Input: part model. Units: mm. Frame: model coordinates. Face numbers are marked on the shaded views. A direction names the side the tool comes from. Round coordinates to 2 decimals unless told otherwise and drop trailing zeros. Loops run counter-clockwise (first coordinate to the right, second up) from the corner with the lowest first, then second, coordinate; pieces in that order, holes last. Notation, with made-up numbers: (10, -38) -> (53, -38) arc R23 cw to (53, -11) -> close; hole circle Ø11 at (84, -30). An arc over 180 degrees is marked (long way). Answer as a JSON object with one key per item and string values. Group by question number.
Item 1: Section query C-C on y = 12.75. Count the separate pieces of the cut face and the enclosed holes in it, and give its area (3 significant figures).
Item 2: Draft query along Z for the marked faces 1, 2 and 3. Return one class per face: released by +Z, released by -Z, zero draft, split by the parting line, or undercut.
Item 3: Material intervals for line 1 (X direction, y = 6.75, z = -22); line 2 (Z direction, x = 18, y = 13.25); line 3 (Z direction, x = -18.5, y = 13.5), sorted ascending. Write a range as [from, to].
Item 4: Set-up query: the marked faces 4 and 5. Return all of +Z, -Z, +X, -X, +Y, -Y with unobstructed straight access to the full face (end or side cutting, diameter ignored); none if empty.
Item 5: Section query D-D on z = 27.5. Return loops of the section in (x, y), and give its area (3 significant figures).
Item 6: Pin query (flat end, axial travel): pin 1 (3.5 mm diameter, centred on x = -31.71, z = -10.3, fed in from +Y); pin 2 (13 mm diameter, centred on x = 17.6, z = -24.22, fed in from +Y); pin 3 (2 mm diameter, centred on x = -7.5, y = 11, fed in from -Z); pin 4 (4 mm diameter, centred on y = 14, z = -7, fed in from +X). Return the tip coordinate at first contact, or that it passes through.
Item 7: Section query A-A on z = 0. Return loops of the section in (x, y) (1 decimal), and give its area (3 significant figures).
Item 8: Section query B-B on x = 0. Return loops of the section in (y, z) (1 decimal), and give its area (3 significant figures).
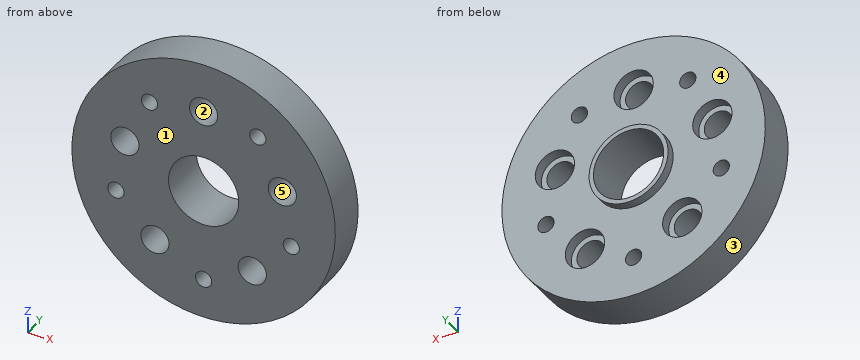
from build123d import *

# Parameters (mm, degrees)
FLANGE_DISC_SKETCH_R              = 47.625
FLANGE_DISC_3_75_DEPTH            = 14.2875
TAPPED_HOLES_SKETCH_R             = 2.930707565
TAPPED_HOLES_5X_ON_BC_2_625_DEPTH = 14.2875
HUB_BOSS_SKETCH_R                 = 14.2875
HUB_BOSS_1_125_DEPTH              = 3.175
CENTER_BORE_SKETCH_R              = 12.7
CENTER_BORE_1_0_DEPTH             = 34.925
COUNTERBORES_SKETCH_R             = 7.112
COUNTERBORES_5X_0_56_DEPTH        = 3.81
BOLT_HOLES_SKETCH_R               = 5.10197716
COUNTERBORED_BOLT_HOLES_5X_DEPTH  = 16.51


with BuildPart() as part:
    # Flange Disc Sketch → Flange Disc Ø3.75 (new body)
    with BuildSketch(Plane(origin=(0, 0, 0), x_dir=(1, 0, 0), z_dir=(0, 1, 0))):
        with Locations(Location((0, 0, 0), (0, 0, 270))):
            Circle(FLANGE_DISC_SKETCH_R)
    extrude(amount=FLANGE_DISC_3_75_DEPTH)

    # Tapped Holes Sketch → Tapped Holes 5x on BC Ø2.625 (cut)
    with BuildSketch(Plane(origin=(0, 14.2875, 0), x_dir=(1, 0, 0), z_dir=(0, 1, 0))):
        with Locations(Location((0, 33.3375, 0), (0, 0, 270))):
            Circle(TAPPED_HOLES_SKETCH_R)
        with Locations(Location((31.705846612, 10.30185405, 0), (0, 0, 270))):
            Circle(TAPPED_HOLES_SKETCH_R)
        with Locations(Location((19.595290848, -26.97060405, 0), (0, 0, 270))):
            Circle(TAPPED_HOLES_SKETCH_R)
        with Locations(Location((-19.595290848, -26.97060405, 0), (0, 0, 270))):
            Circle(TAPPED_HOLES_SKETCH_R)
        with Locations(Location((-31.705846612, 10.30185405, 0), (0, 0, 270))):
            Circle(TAPPED_HOLES_SKETCH_R)
    extrude(amount=-TAPPED_HOLES_5X_ON_BC_2_625_DEPTH, mode=Mode.SUBTRACT)

    # Hub Boss Sketch → Hub Boss Ø1.125 (add)
    with BuildSketch(Plane(origin=(0, 14.2875, 0), x_dir=(1, 0, 0), z_dir=(0, 1, 0))):
        with Locations(Location((0, 0, 0), (0, 0, 270))):
            Circle(HUB_BOSS_SKETCH_R)
    extrude(amount=HUB_BOSS_1_125_DEPTH)

    # Center Bore Sketch → Center Bore Ø1.0 (cut)
    with BuildSketch(Plane(origin=(0, 17.4625, 0), x_dir=(1, 0, 0), z_dir=(0, 1, 0))):
        with Locations(Location((0, 0, 0), (0, 0, 270))):
            Circle(CENTER_BORE_SKETCH_R)
    extrude(amount=-CENTER_BORE_1_0_DEPTH, mode=Mode.SUBTRACT)

    # Counterbores Sketch → Counterbores 5xØ0.56 (cut)
    with BuildSketch(Plane(origin=(0, 14.2875, 0), x_dir=(1, 0, 0), z_dir=(0, 1, 0))):
        with Locations(Location((0, -29.935700362, 0), (0, 0, 270))):
            Circle(COUNTERBORES_SKETCH_R)
        with Locations(Location((-28.470542899, -9.25064015, 0), (0, 0, 270))):
            Circle(COUNTERBORES_SKETCH_R)
        with Locations(Location((-17.59576319, 24.218490331, 0), (0, 0, 270))):
            Circle(COUNTERBORES_SKETCH_R)
        with Locations(Location((17.59576319, 24.218490331, 0), (0, 0, 270))):
            Circle(COUNTERBORES_SKETCH_R)
        with Locations(Location((28.470542899, -9.25064015, 0), (0, 0, 270))):
            Circle(COUNTERBORES_SKETCH_R)
    extrude(amount=-COUNTERBORES_5X_0_56_DEPTH, mode=Mode.SUBTRACT)

    # Bolt Holes Sketch → Counterbored Bolt Holes 5x (cut)
    with BuildSketch(Plane(origin=(0, 10.4775, 0), x_dir=(1, 0, 0), z_dir=(0, 1, 0))):
        with Locations(Location((0, -29.935700362, 0), (0, 0, 270))):
            Circle(BOLT_HOLES_SKETCH_R)
        with Locations(Location((-28.470542899, -9.25064015, 0), (0, 0, 270))):
            Circle(BOLT_HOLES_SKETCH_R)
        with Locations(Location((-17.59576319, 24.218490331, 0), (0, 0, 270))):
            Circle(BOLT_HOLES_SKETCH_R)
        with Locations(Location((17.59576319, 24.218490331, 0), (0, 0, 270))):
            Circle(BOLT_HOLES_SKETCH_R)
        with Locations(Location((28.470542899, -9.25064015, 0), (0, 0, 270))):
            Circle(BOLT_HOLES_SKETCH_R)
    extrude(amount=-COUNTERBORED_BOLT_HOLES_5X_DEPTH, mode=Mode.SUBTRACT)


solid = part.part
Solved:
{
 "1": {"separate pieces": "1", "enclosed holes": "11", "area": "5,690 mm²"},
 "2": {"face 1": "zero draft", "face 2": "undercut", "face 3": "split by the parting line"},
 "3": {"line 1": "[-42.24, -22.19], [-13, 13], [22.19, 42.24]", "line 2": "[-44.09, -31.32], [-17.12, 24.51], [29.43, 44.09]", "line 3": "[-43.88, -31.27], [-17.16, 24.25], [29.69, 43.88]"},
 "4": {"face 4": "+Y", "face 5": "+Y, -Y"},
 "5": {"outline": "(-38.88, 0) -> (-22.48, 0) -> (-22.48, 14.29) -> (-38.88, 14.29) -> close; (-16.71, 0) -> (-4.48, 0) -> (-4.48, 10.48) -> (-6.68, 10.48) -> (-6.68, 14.29) -> (-16.71, 14.29) -> close; (4.48, 0) -> (16.71, 0) -> (16.71, 14.29) -> (6.68, 14.29) -> (6.68, 10.48) -> (4.48, 10.48) -> close; (22.48, 0) -> (38.88, 0) -> (38.88, 14.29) -> (22.48, 14.29) -> close", "area": "801 mm²"},
 "6": {"pin 1": "through", "pin 2": "y = 10.48", "pin 3": "z = -47.18", "pin 4": "x = 47.36"},
 "7": {"outline": "(-47.6, 0) -> (-12.7, 0) -> (-12.7, 17.5) -> (-14.3, 17.5) -> (-14.3, 14.3) -> (-47.6, 14.3) -> close; (12.7, 0) -> (47.6, 0) -> (47.6, 14.3) -> (14.3, 14.3) -> (14.3, 17.5) -> (12.7, 17.5) -> close", "area": "1,010 mm²"},
 "8": {"outline": "(0, -47.6) -> (14.3, -47.6) -> (14.3, -36.3) -> (0, -36.3) -> close; (0, -30.4) -> (14.3, -30.4) -> (14.3, -14.3) -> (17.5, -14.3) -> (17.5, -12.7) -> (0, -12.7) -> close; (0, 12.7) -> (17.5, 12.7) -> (17.5, 14.3) -> (14.3, 14.3) -> (14.3, 22.8) -> (10.5, 22.8) -> (10.5, 24.8) -> (0, 24.8) -> close; (0, 35) -> (10.5, 35) -> (10.5, 37) -> (14.3, 37) -> (14.3, 47.6) -> (0, 47.6) -> close", "area": "763 mm²"}
}
